```python
from build123d import *
from OCP.BRepFilletAPI import BRepFilletAPI_MakeChamfer

# Parameters (mm, degrees)
SKETCH1_R           = 110
BOSS_EXTRUDE1_DEPTH = 25
SKETCH2_R           = 123
SKETCH2_R_2         = 110
CUT_EXTRUDE2_DEPTH  = 2
CHAMFER1_SIZE       = 7
CHAMFER1_SIZE2      = 10
CHAMFER2_SIZE       = 10
CHAMFER2_SIZE2      = 7


with BuildPart() as part:
    # Sketch1 → Boss-Extrude1 (new body)
    with BuildSketch(Plane.XY):
        with BuildLine():
            Line((-120.85, 0), (120.85, 0))
            Line((120.85, 0), (170.370762123, 257.196746905))
            ThreePointArc((170.370762123, 257.196746905), (0, 463.5), (-170.370762123, 257.196746905))
            Line((-170.370762123, 257.196746905), (-120.85, 0))
        make_face()
        with Locations((0, 290)):
            Circle(SKETCH1_R, mode=Mode.SUBTRACT)
    extrude(amount=BOSS_EXTRUDE1_DEPTH)

    # Sketch2 → Cut-Extrude2 (cut)
    with BuildSketch(Plane.XY):
        with Locations((0, 290)):
            Circle(SKETCH2_R)
        with Locations((0, 290)):
            Circle(SKETCH2_R_2, mode=Mode.SUBTRACT)
    extrude(amount=CUT_EXTRUDE2_DEPTH, mode=Mode.SUBTRACT)

    # Chamfer1
    chamfer1_edges = [part.edges().sort_by_distance(p)[0] for p in [
        (0, 463.5, 0),
        (145.610381062, 128.598373453, 0),
        (0, 0, 0),
        (-145.610381062, 128.598373453, 0),
    ]]
    chamfer1_side = [part.faces().sort_by_distance(p)[0] for p in [
        (-139.924807111, 129.693076082, 0),
    ]]
    chamfer(chamfer1_edges, length=CHAMFER1_SIZE, length2=CHAMFER1_SIZE2, reference=chamfer1_side[0])

    # Chamfer2: one chamfer whose edges measure the first distance from different faces: ONE call of the kernel's chamfer builder (chamfer() names one face for all edges)
    chamfer2_edges_1 = [part.edges().sort_by_distance(p)[0] for p in [
        (145.610381062, 128.598373453, 25),
    ]]
    chamfer2_side_1 = [part.faces().sort_by_distance(p)[0] for p in [
        (145.610381062, 128.598373453, 17.5),
    ]]
    chamfer2_edges_2 = [part.edges().sort_by_distance(p)[0] for p in [
        (0, 463.5, 25),
    ]]
    chamfer2_side_2 = [part.faces().sort_by_distance(p)[0] for p in [
        (0, 463.5, 17.5),
    ]]
    chamfer2_edges_3 = [part.edges().sort_by_distance(p)[0] for p in [
        (-145.610381062, 128.598373453, 25),
    ]]
    chamfer2_side_3 = [part.faces().sort_by_distance(p)[0] for p in [
        (-145.610381062, 128.598373453, 17.5),
    ]]
    chamfer2_edges_4 = [part.edges().sort_by_distance(p)[0] for p in [
        (0, 0, 25),
    ]]
    chamfer2_side_4 = [part.faces().sort_by_distance(p)[0] for p in [
        (0, 0, 17.5),
    ]]
    chamfer2 = BRepFilletAPI_MakeChamfer(part.part.solid().wrapped)
    for e in chamfer2_edges_1:
        chamfer2.Add(CHAMFER2_SIZE, CHAMFER2_SIZE2, e.wrapped, chamfer2_side_1[0].wrapped)  # the first distance lies on this face
    for e in chamfer2_edges_2:
        chamfer2.Add(CHAMFER2_SIZE, CHAMFER2_SIZE2, e.wrapped, chamfer2_side_2[0].wrapped)  # the first distance lies on this face
    for e in chamfer2_edges_3:
        chamfer2.Add(CHAMFER2_SIZE, CHAMFER2_SIZE2, e.wrapped, chamfer2_side_3[0].wrapped)  # the first distance lies on this face
    for e in chamfer2_edges_4:
        chamfer2.Add(CHAMFER2_SIZE, CHAMFER2_SIZE2, e.wrapped, chamfer2_side_4[0].wrapped)  # the first distance lies on this face
    add(Compound.cast(chamfer2.Shape()), mode=Mode.REPLACE)


solid = part.part
```
Verification items for the finished model (mm, model axes). A direction names the side the tool comes from. Give positions to 0.01 mm unless a question says otherwise; leave off trailing zeros. Loops run counter-clockwise (first coordinate to the right, second up) from the corner with the lowest first, then second, coordinate; pieces in that order, holes last. Notation, with made-up numbers: M 69,26 L 113,26 A19 cw 113,54 Z; hole C 10,66 d8. An arc over 180 degrees is marked long. Return JSON: item names as keys, results as strings.
1) Tool access check on faces 1 (the flat face through (-92, 227, 2)), 2 (the cylindrical face through (-14.32, 399.064, 13.339)). Record the directions out of +Z, -Z, +X, -X, +Y, -Y that give a thin tool (end or side, any length) a straight path to the whole face; none if there is none.
Findings:
{"face 1": "-Z", "face 2": "+Z, -Z"}
2) Material ranges on L1, parallel to X at y = 339.5, z = 17.25; L2, parallel to Y at x = 0, z = 0.65 (3 decimals); L3, parallel to Y at x = 0, z = 0.95 (3 decimals), recorded low to high. Write a range as [from, to].
Findings:
{"L1": "x = [-164.64, -98.23], [98.23, 164.64]", "L2": "y = [6.545, 167], [413, 456.955]", "L3": "y = [6.335, 167], [413, 457.165]"}
3) Gauge pin test, flat ends, axial feed: P1, Ø4, axis at y = 363.5, z = 21, coming from the +X side; P2, Ø2, axis at x = 84, z = 3.5, coming from the +Y side; P3, Ø4, axis at y = 314.5, z = 9, coming from the +X side. Record the tip position at first contact, or that the pin passes through.
Findings:
{"P1": "stops at x = 154.33", "P2": "stops at y = 437.57", "P3": "stops at x = 172"}
4) Mould release check, pull along X, two halves, no side actions. Record for faces 3 (the flat face through (145.264, 126.798, 12.465)), 4 (the cylindrical face through (4.277, 463.447, 12.465)), 5 (the cylindrical face through (-16.012, 411.953, 0.986)): released by +X, released by -X, zero draft, split by the parting line, or undercut.
Findings:
{"face 3": "released by +X", "face 4": "split by the parting line", "face 5": "undercut"}
5) Section check B-B, the plane x = 0. Enter the section's corners in (y, z), and give its area (3 significant figures).
Findings:
{"outline": "M 0,10 L 7,0 L 167,0 L 167,2 L 180,2 L 180,25 L 7,25 L 0,15 Z; M 400,2 L 413,2 L 413,0 L 456.5,0 L 463.5,10 L 463.5,15 L 456.5,25 L 400,25 Z", "area": "5,900 mm2"}
6) Section check C-C, the plane y = 131. Enter the section's corners in (x, z).
Findings:
{"outline": "M -146.07,10 L -138.94,0 L 138.94,0 L 146.07,10 L 146.07,15 L 138.94,25 L -138.94,25 L -146.07,15 Z"}
7) Section check A-A, the plane y = 290. Enter the section's corners in (x, z).
Findings:
{"outline": "M -173.5,10 L -166.5,0 L -123,0 L -123,2 L -110,2 L -110,25 L -166.5,25 L -173.5,15 Z; M 110,2 L 123,2 L 123,0 L 166.5,0 L 173.5,10 L 173.5,15 L 166.5,25 L 110,25 Z"}
